from build123d import *

# Parameters (mm, degrees)
SKETCH1_W           = 600
SKETCH1_H           = 400
BOSS_EXTRUDE1_DEPTH = 4
SHELL1_T            = -2
SKETCH2_R           = 5.5
CUT_EXTRUDE1_DEPTH  = 4


with BuildPart() as part:
    # Sketch1 → Boss-Extrude1 (new body)
    with BuildSketch(Plane(origin=(0, 0, 0), x_dir=(1, 0, 0), z_dir=(0, 1, 0))):
        Rectangle(SKETCH1_W, SKETCH1_H)
    extrude(amount=BOSS_EXTRUDE1_DEPTH)

    # Shell1
    shell1_openings = [part.faces().sort_by_distance(p)[0] for p in [
        (0, 0, 0),
    ]]
    offset(amount=SHELL1_T, openings=shell1_openings, kind=Kind.INTERSECTION)

    # Sketch2 → Cut-Extrude1 (cut)
    with BuildSketch(Plane(origin=(0, 4, 0), x_dir=(1, 0, 0), z_dir=(0, 1, 0))):
        with Locations(Location((-275, 175, 0), (0, 0, 270))):
            Circle(SKETCH2_R)
        with Locations(Location((275, 175, 0), (0, 0, 270))):
            Circle(SKETCH2_R)
        with Locations(Location((275, -175, 0), (0, 0, 270))):
            Circle(SKETCH2_R)
        with Locations(Location((-275, -175, 0), (0, 0, 270))):
            Circle(SKETCH2_R)
    extrude(amount=-CUT_EXTRUDE1_DEPTH, mode=Mode.SUBTRACT)


solid = part.part
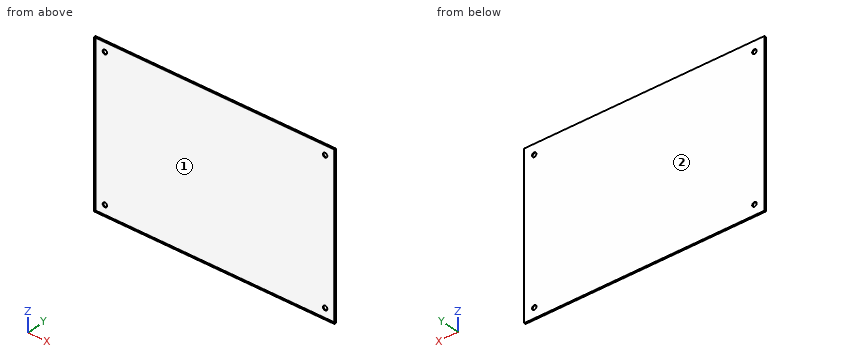
Design review of the part built by this model. Coordinates are the model's own, in mm. Face numbers are marked on the shaded views. Coordinates: 2 decimals unless noted, no trailing zeros. Loops run counter-clockwise (first coordinate to the right, second up) from the corner with the lowest first, then second, coordinate; pieces in that order, holes last.
Item 1: Wall thickness on L1, parallel to Z at x = -275, y = 3.3; L2, parallel to X at y = 3.3, z = 175; L3, parallel to X at y = 0.8, z = 145: over which ranges is each line inside the solid? List them lowest first.
Completed:
L1: z = -200 to -180.5, -169.5 to 169.5, 180.5 to 200
L2: x = -300 to -280.5, -269.5 to 269.5, 280.5 to 300
L3: x = -300 to -298, 298 to 300
Item 2: Add section A-A (y = 0.8). Write out the cut boundary in (x, z), and give its area (3 significant figures).
Completed:
outline: (-300, -200) - (300, -200) - (300, 200) - (-300, 200) - close; hole (-298, -198) - (298, -198) - (298, 198) - (-298, 198) - close
area: 3,980 mm2
Item 3: Clearance check with flat-ended pins moving along their axes: pin 1 (10 mm diameter, centred on x = -69, z = -107.5, fed in from -Y); pin 2 (10 mm diameter, centred on x = 275, z = -175, fed in from +Y). State where each tip first meets the part, or that it passes through.
Completed:
pin 1: stops at y = 2
pin 2: passes through
Item 4: Draft analysis for pull direction Y (two halves, no side actions). For the marked faces 1 and 2, state which applies: pulls with the +Y half, pulls with the -Y half, needs draft (parallel to the pull), parting line crosses it, or undercut.
Completed:
face 1: pulls with the -Y half
face 2: pulls with the +Y half
Item 5: Add section C-C (z = 15). Write out the cut boundary in (x, y).
Completed:
outline: (-300, 0) - (-298, 0) - (-298, 2) - (298, 2) - (298, 0) - (300, 0) - (300, 4) - (-300, 4) - close
Item 6: Add section B-B (x = 185). Write out the cut boundary in (y, z).
Completed:
outline: (0, -200) - (4, -200) - (4, 200) - (0, 200) - (0, 198) - (2, 198) - (2, -198) - (0, -198) - close
